Check sheet for the modelled part. Datum: model origin and axes. Units: mm. Face numbers are marked on the shaded views. A direction names the side the tool comes from. Coordinates: 2 decimals unless noted, no trailing zeros. Write each loop counter-clockwise with the first axis right and the second up, starting at its lowest first coordinate (ties: lowest second). Pieces come first, ordered by that corner, then holes. Notation, with made-up numbers: (2, 33.5) - (58, 33.5) arc R28 ccw to (58, 70.5) - close; hole circle Ø8 at (1, 89). An arc over 180 degrees is marked (long way). Answer as CSV lines item,"result". Start each with the question number.
from build123d import *

# Parameters (mm, degrees)
L_BRACKET_BODY_DEPTH          = 110
VERTICAL_LEG_SLOTS_3X10_DEPTH = 110
BASE_HOLES_SKETCH_R           = 7
BASE_MOUNTING_HOLES_DEPTH     = 110
INNER_CORNER_FILLET_R5_R      = 5


with BuildPart() as part:
    # Bracket L-Profile Sketch → L-Bracket Body (new body)
    with BuildSketch(Plane(origin=(0, 0, 0), x_dir=(0, 0, -1), z_dir=(1, 0, 0))):
        Polygon((0, 0), (0, 75), (14, 75), (14, 10), (70, 10), (70, 0), align=None)
    extrude(amount=-L_BRACKET_BODY_DEPTH)

    # Vertical Leg Slots Sketch → Vertical Leg Slots 3x10 (cut)
    with BuildSketch(Plane(origin=(0, 0, -14), x_dir=(-1, 0, 0), z_dir=(0, 0, -1))):
        with BuildLine():
            Line((15, 65), (15, 30))
            ThreePointArc((15, 30), (20, 25), (25, 30))
            Line((25, 30), (25, 65))
            ThreePointArc((25, 65), (20, 70), (15, 65))
        make_face()
        with BuildLine():
            Line((50, 65), (50, 30))
            ThreePointArc((50, 30), (55, 25), (60, 30))
            Line((60, 30), (60, 65))
            ThreePointArc((60, 65), (55, 70), (50, 65))
        make_face()
        with BuildLine():
            Line((85, 65), (85, 30))
            ThreePointArc((85, 30), (90, 25), (95, 30))
            Line((95, 30), (95, 65))
            ThreePointArc((95, 65), (90, 70), (85, 65))
        make_face()
    extrude(amount=-VERTICAL_LEG_SLOTS_3X10_DEPTH, mode=Mode.SUBTRACT)

    # Base Holes Sketch → Base Mounting Holes (cut)
    with BuildSketch(Plane(origin=(0, 10, 0), x_dir=(1, 0, 0), z_dir=(0, 1, 0))):
        with Locations(Location((-95, 55, 0), (0, 0, 270))):
            Circle(BASE_HOLES_SKETCH_R)
        with Locations(Location((-15, 55, 0), (0, 0, 270))):
            Circle(BASE_HOLES_SKETCH_R)
        with Locations(Location((-15, 27, 0), (0, 0, 270))):
            Circle(BASE_HOLES_SKETCH_R)
        with Locations(Location((-95, 27, 0), (0, 0, 270))):
            Circle(BASE_HOLES_SKETCH_R)
        with BuildLine():
            Line((-75, 49), (-35, 49))
            ThreePointArc((-35, 49), (-28, 42), (-35, 35))
            Line((-35, 35), (-75, 35))
            ThreePointArc((-75, 35), (-82, 42), (-75, 49))
        make_face()
    extrude(amount=-BASE_MOUNTING_HOLES_DEPTH, mode=Mode.SUBTRACT)

    # Inner Corner Fillet R5
    inner_corner_fillet_r5_edges = [part.edges().sort_by_distance(p)[0] for p in [
        (-55, 10, -14),
    ]]
    fillet(inner_corner_fillet_r5_edges, radius=INNER_CORNER_FILLET_R5_R)


solid = part.part
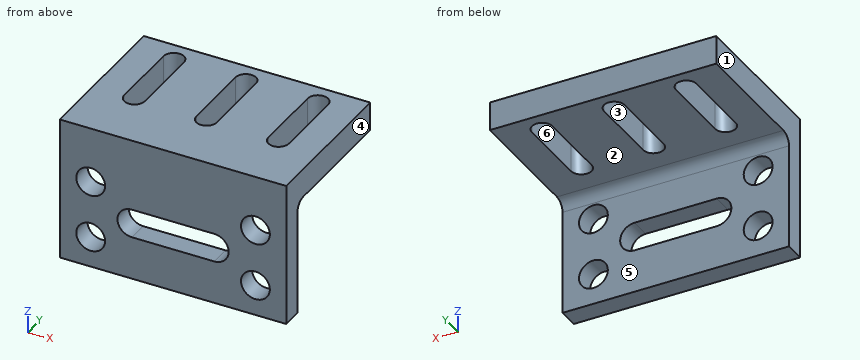
(1) Release check for a two-part mould opening along Y. For the marked faces 4, 5 and 6 record: pulls with the +Y half, pulls with the -Y half, needs draft (parallel to the pull), parting line crosses it, or undercut.
(2) Cross-section at A-A on x = -48.5. Record the boundary of the cut face in (y, z).
(3) Tool access check on the marked faces 1, 2 and 3. Record the directions out of +Z, -Z, +X, -X, +Y, -Y that give a thin tool (end or side, any length) a straight path to the whole face; none if there is none.
(4) Material ranges on probe 1 along X at (y, z) = (5.5, -55); probe 2 along Z at (x, y) = (-81.5, 66); probe 3 along Y at (x, z) = (-22.5, -42.5), recorded low to high. Write a range as from..to.
(5) Cross-section at B-B on z = -42. Record the boundary of the cut face in (x, y), plus the area to 3 significant figures.
(6) Cross-section at C-C on z = -55. Record the boundary of the cut face in (x, y).
(7) Cross-section at D-D on z = -8.5. Record the boundary of the cut face in (x, y), plus the area to 3 significant figures.
(8) Go/stop test with flat-tipped pins: P1, Ø4, axis at x = -73.5, y = 40.5, coming from the -Z side; P2, Ø18, axis at x = -95, z = -55, coming from the +Y side; P3, Ø12.5, axis at x = -95, z = -27, coming from the +Y side. Record where each tip stops, or that it passes through.
Checked values:
1,face 4,"needs draft"
1,face 5,"pulls with the +Y half"
1,face 6,"undercut"
2,outline,"(0, -70) - (10, -70) - (10, -49) - (0, -49) - close; (0, -35) - (10, -35) - (10, -19) arc R5 cw to (15, -14) - (75, -14) - (75, 0) - (0, 0) - close"
3,face 1,"+Z, -Z, -X, +Y, -Y"
3,face 2,"-Z, +X, -X, +Y"
3,face 3,"+Z, -Z"
4,probe 1,"-110..-102, -88..-22, -8..0"
4,probe 2,"-14..0"
4,probe 3,"0..10"
5,outline,"(-110, 0) - (-82, 0) - (-82, 10) - (-110, 10) - close; (-28, 0) - (0, 0) - (0, 10) - (-28, 10) - close"
5,area,"560 mm^2"
6,outline,"(-110, 0) - (-102, 0) - (-102, 10) - (-110, 10) - close; (-88, 0) - (-22, 0) - (-22, 10) - (-88, 10) - close; (-8, 0) - (0, 0) - (0, 10) - (-8, 10) - close"
7,outline,"(-110, 0) - (0, 0) - (0, 75) - (-110, 75) - close; hole (-95, 30) arc R5 ccw to (-85, 30) - (-85, 65) arc R5 ccw to (-95, 65) - close; hole (-60, 30) arc R5 ccw to (-50, 30) - (-50, 65) arc R5 ccw to (-60, 65) - close; hole (-25, 30) arc R5 ccw to (-15, 30) - (-15, 65) arc R5 ccw to (-25, 65) - close"
7,area,"6,960 mm^2"
8,P1,"z = -14"
8,P2,"y = 10"
8,P3,"through"
